Check sheet for the modelled part. Datum: model origin and axes. Units: mm. A direction names the side the tool comes from. Coordinates: 2 decimals unless noted, no trailing zeros. Order: outer loops, then holes, each group sorted by start corner. A loop starts at its lowest first (then second) coordinate and runs counter-clockwise, first axis right, second up. Notation, with made-up numbers: M 16,-5.5 L 27,-5.5 A20 cw 27,14.5 Z; hole C -29,72 d10. An arc over 180 degrees is marked long. Answer in a Markdown table with one row per item. Add a question column.
from build123d import *

# Parameters (mm, degrees)
SKETCH_1_W          = 170
SKETCH_1_H          = 75
EXTRUDE_1_DEPTH     = 10
CHAMFER_1_SIZE      = 5
SKETCH_2_R          = 2.75
CUT_EXTRUDE_1_DEPTH = 15


with BuildPart() as part:
    # 草图1 → 凸台-拉伸1 (new body)
    with BuildSketch(Plane(origin=(0, 0, 0), x_dir=(1, 0, 0), z_dir=(0, 1, 0))):
        Rectangle(SKETCH_1_W, SKETCH_1_H)
    extrude(amount=EXTRUDE_1_DEPTH)

    # 倒角1
    chamfer_1_edges = [part.edges().sort_by_distance(p)[0] for p in [
        (85, 5, 37.5),
        (-85, 5, 37.5),
        (-85, 5, -37.5),
        (85, 5, -37.5),
    ]]
    chamfer(chamfer_1_edges, length=CHAMFER_1_SIZE)

    # 草图2 → 切除-拉伸1 (cut)
    with BuildSketch(Plane(origin=(0, 10, 0), x_dir=(1, 0, 0), z_dir=(0, 1, 0))):
        with Locations(Location((15, 25, 0), (0, 0, 270))):
            Circle(SKETCH_2_R)
        with Locations(Location((45, 25, 0), (0, 0, 270))):
            Circle(SKETCH_2_R)
        with Locations(Location((75, 25, 0), (0, 0, 270))):
            Circle(SKETCH_2_R)
        with Locations(Location((15, -22.5, 0), (0, 0, 270))):
            Circle(SKETCH_2_R)
        with Locations(Location((45, -22.5, 0), (0, 0, 270))):
            Circle(SKETCH_2_R)
        with Locations(Location((75, -22.5, 0), (0, 0, 270))):
            Circle(SKETCH_2_R)
        with BuildLine():
            Line((-72.25, 29.75), (-72.25, 20.25))
            ThreePointArc((-72.25, 20.25), (-75, 17.5), (-77.75, 20.25))
            Line((-77.75, 20.25), (-77.75, 29.75))
            ThreePointArc((-77.75, 29.75), (-75, 32.5), (-72.25, 29.75))
        make_face()
        with BuildLine():
            Line((-42.25, 29.75), (-42.25, 20.25))
            ThreePointArc((-42.25, 20.25), (-45, 17.5), (-47.75, 20.25))
            Line((-47.75, 20.25), (-47.75, 29.75))
            ThreePointArc((-47.75, 29.75), (-45, 32.5), (-42.25, 29.75))
        make_face()
        with BuildLine():
            Line((-72.25, -17.75), (-72.25, -27.25))
            ThreePointArc((-72.25, -27.25), (-75, -30), (-77.75, -27.25))
            Line((-77.75, -27.25), (-77.75, -17.75))
            ThreePointArc((-77.75, -17.75), (-75, -15), (-72.25, -17.75))
        make_face()
        with BuildLine():
            Line((-42.25, -17.75), (-42.25, -27.25))
            ThreePointArc((-42.25, -27.25), (-45, -30), (-47.75, -27.25))
            Line((-47.75, -27.25), (-47.75, -17.75))
            ThreePointArc((-47.75, -17.75), (-45, -15), (-42.25, -17.75))
        make_face()
    extrude(amount=-CUT_EXTRUDE_1_DEPTH, mode=Mode.SUBTRACT)


solid = part.part
1. Set-up check for faces 4 (the flat face through (-72.25, 5, -25)), 5 (the flat face through (-1, 5, 37.5)): record each of +Z, -Z, +X, -X, +Y, -Y from which the full face is reachable in a straight line by a thin tool's end or side.
2. Scan lines: line 1 (X direction, y = 4.75, z = -25); line 2 (X direction, y = 2, z = 18.5); line 3 (X direction, y = 9.25, z = 24.5). Record each from-to range of solid material in increasing order.
3. Release check for a two-part mould opening along Z. For faces 1 (the cylindrical face through (46.859, 5.07, -27.027)), 2 (the flat face through (-1, 5, -37.5)), 3 (the flat face through (-82.5, 4.9, 35)) record: released by +Z, released by -Z, zero draft, split by the parting line, or undercut.
4. Section check B-B on x = 75. Enter the section's corners in (y, z), then the cut area to 3 significant figures.
5. Section check A-A on y = 8.5. State how many separate pieces and enclosed holes the cut face has, then the cut area to 3 significant figures.
6. Section check C-C on z = 22.5. Enter the section's corners in (x, y), then the cut area to 4 significant figures.
7. Go/stop test with a flat-tipped pin: pin 1 Ø3.5 at (x, z) = (15, 22.5) entering from +Y. Record where the tip stops, or that it passes through.
Result sheet:
| question | item | result |
|---|---|---|
| 1 | face 4 | +Y, -Y |
| 1 | face 5 | +Z, +X, -X, +Y, -Y |
| 2 | line 1 | -85 to -77.75, -72.25 to -47.75, -42.25 to 12.25, 17.75 to 42.25, 47.75 to 72.25, 77.75 to 85 |
| 2 | line 2 | -85 to -77.75, -72.25 to -47.75, -42.25 to 85 |
| 2 | line 3 | -85 to -77.75, -72.25 to -47.75, -42.25 to 13.11, 16.89 to 43.11, 46.89 to 73.11, 76.89 to 85 |
| 3 | face 1 | undercut |
| 3 | face 2 | released by -Z |
| 3 | face 3 | released by +Z |
| 4 | outline | M 0,-37.5 L 10,-37.5 L 10,-27.75 L 0,-27.75 Z; M 0,-22.25 L 10,-22.25 L 10,19.75 L 0,19.75 Z; M 0,25.25 L 10,25.25 L 10,37.5 L 0,37.5 Z |
| 4 | area | 640 mm^2 |
| 5 | separate pieces | 1 |
| 5 | enclosed holes | 10 |
| 5 | area | 12,300 mm^2 |
| 6 | outline | M -85,0 L -77.75,0 L -77.75,10 L -85,10 Z; M -72.25,0 L -47.75,0 L -47.75,10 L -72.25,10 Z; M -42.25,0 L 12.25,0 L 12.25,10 L -42.25,10 Z; M 17.75,0 L 42.25,0 L 42.25,10 L 17.75,10 Z; M 47.75,0 L 72.25,0 L 72.25,10 L 47.75,10 Z; M 77.75,0 L 85,0 L 85,10 L 77.75,10 Z |
| 6 | area | 1,425 mm^2 |
| 7 | pin 1 | through |
